Part model, mm, in its own coordinate system. Coordinates: 2 decimals unless noted, no trailing zeros. Loops run counter-clockwise (first coordinate to the right, second up) from the corner with the lowest first, then second, coordinate; pieces in that order, holes last. Notation, with made-up numbers: M -2.75,-35 L 53.25,-35 A21 ccw 53.25,-4 Z; hole C 79,-24 d4. An arc over 180 degrees is marked long. Answer as a JSON object with one key per item and string values. Group by question number.
1. Saw through at B-B on z = 19. Write the cut outline in (x, y).
2. Drop flat-ended pins along their axis: pin 1 Ø10 at (x, y) = (432, 21) entering from +Z; pin 2 Ø6 at (x, z) = (142.5, 21.5) entering from -Y; pin 3 Ø2.5 at (x, z) = (732.5, 2) entering from -Y; pin 4 Ø6 at (x, z) = (168, 27) entering from +Y. Give the stop position or say it passes through.
3. Drill centre lines: L1, parallel to Y at x = 491, z = 20; L2, parallel to X at y = 2, z = 30.5. Where is each one in solid material? Low to high.
4. Saw through at A-A on x = 393. Write the cut outline in (y, z).
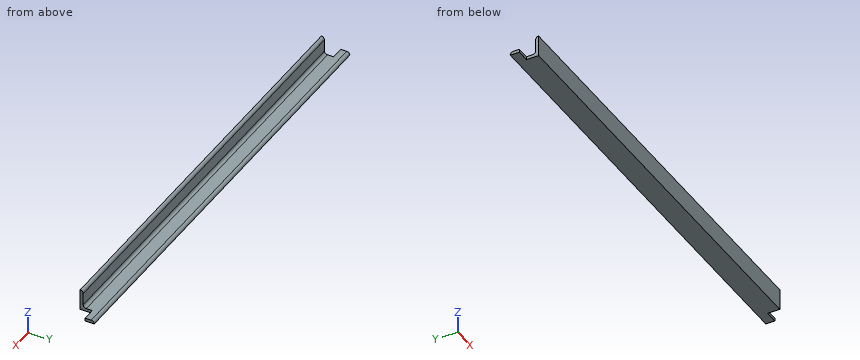
from build123d import *

# Parameters (mm, degrees)
ANGLE_IRON_35_X_35_X_5_1_DEPTH = 747
SKETCH2_W                      = 21
SKETCH2_H                      = 20
CUT_EXTRUDE1_DEPTH             = 749.638096813


with BuildPart() as part:
    # Sketch11 → Angle Iron 35 X 35 X 5(1) (new body)
    with BuildSketch(Plane.YZ):
        with BuildLine():
            Line((0, 0), (0, 35))
            ThreePointArc((0, 35), (3.535533906, 33.535533906), (5, 30))
            Line((5, 30), (5, 10))
            ThreePointArc((5, 10), (6.464466094, 6.464466094), (10, 5))
            Line((10, 5), (30, 5))
            ThreePointArc((30, 5), (33.535533906, 3.535533906), (35, 0))
            Line((35, 0), (0, 0))
        make_face()
    extrude(amount=ANGLE_IRON_35_X_35_X_5_1_DEPTH)

    # Sketch2 → Cut-Extrude1 (cut, through all)
    with BuildSketch(Plane(origin=(0, 0, 0), x_dir=(-1, 0, 0), z_dir=(0, 0, -1))):
        with Locations((-10.5, 10)):
            Rectangle(SKETCH2_W, SKETCH2_H)
        with Locations((-736.5, 10)):
            Rectangle(SKETCH2_W, SKETCH2_H)
    extrude(amount=-CUT_EXTRUDE1_DEPTH, mode=Mode.SUBTRACT)


solid = part.part
Outcome:
{
 "1": {"outline": "M 21,0 L 726,0 L 726,5 L 21,5 Z"},
 "2": {"pin 1": "stops at z = 5", "pin 2": "stops at y = 0", "pin 3": "stops at y = 20", "pin 4": "stops at y = 5"},
 "3": {"L1": "y = 0 to 5", "L2": "x = 21 to 726"},
 "4": {"outline": "M 0,0 L 35,0 A5 ccw 30,5 L 10,5 A5 cw 5,10 L 5,30 A5 ccw 0,35 Z"}
}
